Read the model definition and answer for the solid it produces. Units are mm, in the model's axes. A direction names the side the tool comes from. Round coordinates to 2 decimals unless told otherwise and drop trailing zeros. Loops run counter-clockwise (first coordinate to the right, second up) from the corner with the lowest first, then second, coordinate; pieces in that order, holes last. Notation, with made-up numbers: (-21, -15.5) - (3, -15.5) arc R26 cw to (3, 3.5) - close; hole circle Ø1 at (89, 26). An arc over 180 degrees is marked (long way). Use CSV: the item, a comma, the result in double quotes. Start each with the question number.
1. Find section D-D (y = 17.5). Give the vertices of the cut face in (x, z).
2. Find section B-B (x = 124). Give the vertices of the cut face in (y, z).
3. Find section A-A (x = 55). Give the vertices of the cut face in (y, z).
4. Determine the mould class of faces 3 (the flat face through (0, 77, 7)), 4 (the flat face through (198, 0, 7)), 5 (the cylindrical face through (113.51, 168.46, 6.9)) for opening direction X: +X half, -X half, draft (parallel to the pull), parting line (faces both ways), or undercut.
5. Consider line 1 along Y through (x, z) = (55, 10.25); line 2 along Y through (x, z) = (355, 6); line 3 along X through (y, z) = (202, 9.25). Determine where each line is inside the solid, lowest interval first.
6. Find section C-C (z = 6). Give the vertices of the cut face in (x, y).
7. A tool of negligible diameter and unlimited length cuts with its end or side. For faces 1 (the flat face through (25, 190, 7)), 2 (the flat face through (390, 91, 7)), from which of +Z, -Z, +X, -X, +Y, -Y can it reach the whole face along a straight path? Write none if from no direction.
8. Given pin 1 Ø7 at (y, z) = (185.5, 4) entering from -X; pin 2 Ø11 at (x, y) = (55, 17.5) entering from -Z; pin 3 Ø7 at (x, y) = (55, 142.5) entering from +Z, each flat-ended and moving along its own axis, determine where each tip first touches the part or whether it passes through.
from build123d import *

# Parameters (mm, degrees)
SKETCH1_R           = 10.5
BOSS_EXTRUDE1_DEPTH = 14
M10_TAPPED_HOLE1_D  = 8.5
SKETCH4_W           = 25
SKETCH4_H           = 60
CUT_EXTRUDE1_DEPTH  = 448.99107134
CHAMFER1_SIZE       = 10
CUT_EXTRUDE2_DEPTH  = 448.99107134


with BuildPart() as part:
    # Sketch1 → Boss-Extrude1 (new body)
    with BuildSketch(Plane.XY):
        Polygon((0, 220), (315, 220), (390, 170), (390, 0), (0, 0), align=None)
        with Locations((124, 168)):
            Circle(SKETCH1_R, mode=Mode.SUBTRACT)
    extrude(amount=BOSS_EXTRUDE1_DEPTH)

    # M10 Tapped Hole1 (through all)
    with Locations(Plane.XY.offset(14)):
        with Locations((55, 142.5), (55, 17.5), (355, 142.5), (355, 17.5)):
            Hole(M10_TAPPED_HOLE1_D / 2)

    # Sketch4 → Cut-Extrude1 (cut, through all)
    with BuildSketch(Plane.XY.offset(14)):
        with Locations((12.5, 190)):
            Rectangle(SKETCH4_W, SKETCH4_H)
    extrude(amount=-CUT_EXTRUDE1_DEPTH, mode=Mode.SUBTRACT)

    # Chamfer1
    chamfer1_edges = [part.edges().sort_by_distance(p)[0] for p in [
        (25, 220, 7),
        (25, 160, 7),
        (390, 0, 7),
        (0, 0, 7),
    ]]
    chamfer(chamfer1_edges, length=CHAMFER1_SIZE)

    # Sketch5 → Cut-Extrude2 (cut, through all)
    with BuildSketch(Plane.XY.offset(14)):
        Polygon((15, 160), (0, 160), (0, 145), align=None)
    extrude(amount=-CUT_EXTRUDE2_DEPTH, mode=Mode.SUBTRACT)


solid = part.part
Filled sheet:
1,outline,"(0, 0) - (50.75, 0) - (50.75, 14) - (0, 14) - close; (59.25, 0) - (350.75, 0) - (350.75, 14) - (59.25, 14) - close; (359.25, 0) - (390, 0) - (390, 14) - (359.25, 14) - close"
2,outline,"(0, 0) - (157.5, 0) - (157.5, 14) - (0, 14) - close; (178.5, 0) - (220, 0) - (220, 14) - (178.5, 14) - close"
3,outline,"(0, 0) - (13.25, 0) - (13.25, 14) - (0, 14) - close; (21.75, 0) - (138.25, 0) - (138.25, 14) - (21.75, 14) - close; (146.75, 0) - (220, 0) - (220, 14) - (146.75, 14) - close"
4,face 3,"-X half"
4,face 4,"draft"
4,face 5,"undercut"
5,line 1,"y = 0 to 13.25, 21.75 to 138.25, 146.75 to 220"
5,line 2,"y = 0 to 13.25, 21.75 to 138.25, 146.75 to 193.33"
5,line 3,"x = 25 to 342"
6,outline,"(0, 10) - (10, 0) - (380, 0) - (390, 10) - (390, 170) - (315, 220) - (35, 220) - (25, 210) - (25, 170) - (0, 145) - close; hole circle Ø8.5 at (55, 17.5); hole circle Ø8.5 at (55, 142.5); hole circle Ø21 at (124, 168); hole circle Ø8.5 at (355, 17.5); hole circle Ø8.5 at (355, 142.5)"
7,face 1,"+Z, -Z, -X, +Y"
7,face 2,"+Z, -Z, +X, +Y, -Y"
8,pin 1,"stops at x = 25"
8,pin 2,"stops at z = 0"
8,pin 3,"passes through"
